Could you check a few things on this model? Use its own coordinates, in mm. Face numbers are marked on the shaded views. A direction names the side the tool comes from. Round coordinates to 2 decimals unless told otherwise and drop trailing zeros. Order: outer loops, then holes, each group sorted by start corner. A loop starts at its lowest first (then second) coordinate and runs counter-clockwise, first axis right, second up. Notation, with made-up numbers: (-14, 62.25) - (-1, 62.25) arc R18 cw to (-1, 82.25) - close; hole circle Ø5 at (84.25, -31.75). An arc over 180 degrees is marked (long way). Return JSON: item names as keys, results as strings. Group by question number.
from build123d import *

# Parameters (mm, degrees)
BOSS_EXTRUDE1_DEPTH      = 9.525
BOSS_EXTRUDE1_DEPTH_BACK = 9.525
SKETCH1_R                = 3.9624
BOSS_EXTRUDE2_DEPTH      = 14.2875
BOSS_EXTRUDE2_DEPTH_BACK = 14.2875
BOSS_EXTRUDE2_START      = -9.525
SKETCH2_R                = 3.175


with BuildPart() as part:
    # Sketch1 → Boss-Extrude1 (new, two sides: drawn at the far end of the back side and taken through both)
    with BuildSketch(Plane.XY.offset(-BOSS_EXTRUDE1_DEPTH_BACK)):
        Circle(SKETCH1_R)
    extrude(amount=BOSS_EXTRUDE1_DEPTH + BOSS_EXTRUDE1_DEPTH_BACK)

    # Sketch2 → Boss-Extrude2 (add, two sides: drawn at the far end of the back side and taken through both)
    with BuildSketch(Plane.XY.offset(9.525).offset(BOSS_EXTRUDE2_START - BOSS_EXTRUDE2_DEPTH_BACK)):
        Circle(SKETCH2_R)
    extrude(amount=BOSS_EXTRUDE2_DEPTH + BOSS_EXTRUDE2_DEPTH_BACK)


solid = part.part
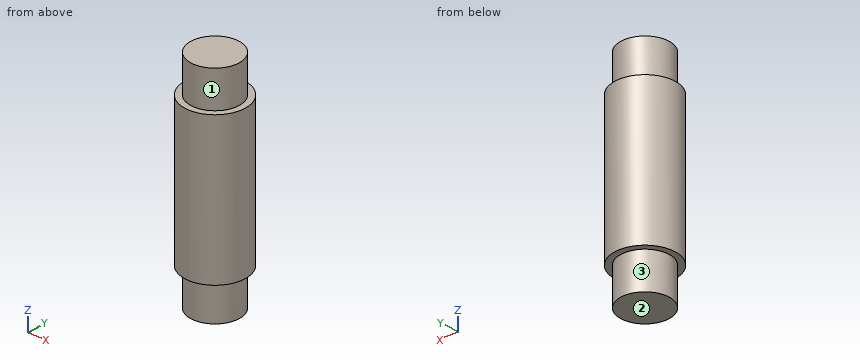
1) I want a section at A-A, the plane x = 0. List the corners of the cut face in (y, z) for me (1 decimal).
2) For the marked faces 1, 2 and 3, which set-ups out of +Z, -Z, +X, -X, +Y, -Y let a thin tool reach every point of the face, with its end or its side?
3) If I drill on line 1 along Z through (x, y) = (-3.25, 2) (3 decimals); line 2 along Y through (x, z) = (3.5, -3.5); line 3 along Y through (x, z) = (-1.75, -1.25), over which ranges is the centre line in solid material (lowest first)? Write a range as from..to.
4) I want a section at C-C, the plane z = 11. List the corners of the cut face in (x, y) for me (3 decimals).
Outcome:
{
 "1": {"outline": "(-4, -9.5) - (-3.2, -9.5) - (-3.2, -14.3) - (3.2, -14.3) - (3.2, -9.5) - (4, -9.5) - (4, 9.5) - (3.2, 9.5) - (3.2, 14.3) - (-3.2, 14.3) - (-3.2, 9.5) - (-4, 9.5) - close"},
 "2": {"face 1": "+Z", "face 2": "-Z, +X, -X, +Y, -Y", "face 3": "-Z"},
 "3": {"line 1": "-9.525..9.525", "line 2": "-1.86..1.86", "line 3": "-3.56..3.56"},
 "4": {"outline": "circle Ø6.35 at (0, 0)"}
}
